The listing builds one solid part. Answer for the finished solid, in the listing's coordinates (mm). A direction names the side the tool comes from. Give positions to 0.01 mm unless a question says otherwise; leave off trailing zeros. Order: outer loops, then holes, each group sorted by start corner. A loop starts at its lowest first (then second) coordinate and runs counter-clockwise, first axis right, second up. Notation, with made-up numbers: (-17.5, -38.5) -> (17.5, -38.5) arc R16 cw to (17.5, -18.5) -> close; hole circle Ø11 at (19, 28.25). An arc over 180 degrees is marked (long way). Answer as a JSON object with one key per item and string values. Group by question number.
```python
from build123d import *

# Parameters (mm, degrees)
HOUSING_BODY_SKETCH_R   = 40
HOUSING_BODY_SKETCH_R_2 = 28
HOUSING_BODY_DEPTH      = 30
MOUNTING_FLANGE_DEPTH   = 25
KEYED_START             = 100
KEYED_HUB_SKETCH_R      = 28
KEYED_HUB_56_DEPTH      = 20
SIDE_RIB_DEPTH          = 20
SLOT_CUT_SKETCH_W       = 30
SLOT_CUT_SKETCH_H       = 10
SLOT_CUT_10X30_DEPTH    = 118.08543889


with BuildPart() as part:
    # Housing Body Sketch → Housing Body (new, symmetric)
    with BuildSketch(Plane(origin=(0, 0, 0), x_dir=(0, 0, -1), z_dir=(1, 0, 0))):
        Circle(HOUSING_BODY_SKETCH_R)
        Circle(HOUSING_BODY_SKETCH_R_2, mode=Mode.SUBTRACT)
    extrude(amount=HOUSING_BODY_DEPTH, both=True)

    # Mounting Flange Sketch → Mounting Flange (add, symmetric)
    with BuildSketch(Plane(origin=(0, 0, 0), x_dir=(0, 0, -1), z_dir=(1, 0, 0))):
        with BuildLine():
            Line((-33.071891388, -22.5), (-50, -22.5))
            Line((-50, -22.5), (-50, -53))
            Line((-50, -53), (50, -53))
            Line((50, -53), (50, 53))
            Line((50, 53), (-50, 53))
            Line((-50, 53), (-50, 22.5))
            Line((-50, 22.5), (-33.071891388, 22.5))
            ThreePointArc((-33.071891388, 22.5), (11.771243445, 38.228756555), (40, 0))
            ThreePointArc((40, 0), (11.771243445, -38.228756555), (-33.071891388, -22.5))
        make_face()
    extrude(amount=MOUNTING_FLANGE_DEPTH, both=True)



with BuildPart() as body_2:
    # Keyed Hub Sketch → Keyed Hub Ø56 (new body)
    with BuildSketch(Plane.XY.offset(KEYED_START)):
        Circle(KEYED_HUB_SKETCH_R)
        with BuildLine():
            Line((-4, 12.369316877), (-4, 15.369316877))
            Line((-4, 15.369316877), (4, 15.369316877))
            Line((4, 15.369316877), (4, 12.369316877))
            ThreePointArc((4, 12.369316877), (0, -13), (-4, 12.369316877))
        make_face(mode=Mode.SUBTRACT)
    extrude(amount=-KEYED_HUB_56_DEPTH)


with BuildPart() as part_1:
    add(part.part)

    add(body_2.part)  # Side Rib merges body 2
    # Side Rib Sketch → Side Rib (add, symmetric)
    with BuildSketch(Plane(origin=(0, 0, 0), x_dir=(0, 0, -1), z_dir=(1, 0, 0))):
        Polygon((-50, 35), (-95, 35), (-95, 17), (-80, 17), (-80, 22.5), (-50, 22.5), align=None)
    side_rib = extrude(amount=SIDE_RIB_DEPTH, both=True)

    # Side Rib Mirror: Side Rib across plane
    add(side_rib.mirror(Plane.ZX))

    # Slot Cut Sketch → Slot Cut 10x30 (cut, through all)
    with BuildSketch(Plane.XY.offset(50)):
        with Locations((0, 48)):
            Rectangle(SLOT_CUT_SKETCH_W, SLOT_CUT_SKETCH_H)
    slot_cut_10x30 = extrude(amount=-SLOT_CUT_10X30_DEPTH, mode=Mode.SUBTRACT)

    # Slot Cut Mirror: Slot Cut 10x30 across plane
    add(slot_cut_10x30.mirror(Plane.ZX), mode=Mode.SUBTRACT)


solid = part_1.part
```
(1) A cutting plane is placed at D-D (y = 18). Determine the outline of the cut face in (x, z), and give its area (3 significant figures).
(2) Find the intervals of material crossed by line 1 along X through (y, z) = (0, 86); line 2 along Z through (x, y) = (-9, -19.5); line 3 along Y through (x, z) = (-11, 57.5), in increasing order. Write a range as [from, to].
(3) Flat-ended cylindrical pins translate along their axes: pin 1 Ø2 at (x, z) = (15.5, 60) entering from -Y; pin 2 Ø15 at (x, z) = (5.5, 13.5) entering from +Y; pin 3 Ø24 at (x, z) = (-2, 6) entering from -Y. Find the tip coordinate at first contact, or state that the pin passes through.
(4) A cutting plane is placed at A-A (y = 0). Determine the outline of the cut face in (x, z), and give its area (3 significant figures).
(5) Which of the six approach directions +Z, -Z, +X, -X, +Y, -Y give full straight-line access (tool end or side, diameter ignored) to faces 1 (the flat face through (0, 43, 1)), 2 (the flat face through (-15, -48, 1)), 3 (the flat face through (0, 31, 95)), 4 (the flat face through (0, -22.5, 57)), 5 (the flat face through (4, 14, 90))?
(6) A cutting plane is placed at C-C (x = 0). Determine the outline of the cut face in (y, z).
(7) For a pull along Y with two mould halves and no side action, classify faces 6 (the flat face through (-20, -53, 1)), 7 (the cylindrical face through (-27.973, 1.231, 92.362)), 8 (the flat face through (-4, 14, 90)), 9 (the flat face through (-30, -8, 27)) as +Y half, -Y half, draft (parallel to the pull), parting line (faces both ways), or undercut.
(8) A cutting plane is placed at B-B (z = 54). Determine the outline of the cut face in (x, y), and give its area (3 significant figures).
Check sheet entries:
{
 "1": {"outline": "(-30, -35.72) -> (-25, -35.72) -> (-25, -50) -> (25, -50) -> (25, -35.72) -> (30, -35.72) -> (30, -21.45) -> (-30, -21.45) -> close; (-30, 21.45) -> (30, 21.45) -> (30, 35.72) -> (-30, 35.72) -> close; (-21.45, 80) -> (21.45, 80) -> (21.45, 100) -> (-21.45, 100) -> close", "area": "3,280 mm2"},
 "2": {"line 1": "x = [-28, -13], [13, 28]", "line 2": "z = [-50, -20.09], [20.09, 34.92], [80, 100]", "line 3": "y = [-35, -22.5], [22.5, 35]"},
 "3": {"pin 1": "stops at y = -35", "pin 2": "stops at y = 43", "pin 3": "stops at y = -43"},
 "4": {"outline": "(-30, -40) -> (-25, -40) -> (-25, -50) -> (25, -50) -> (25, -40) -> (30, -40) -> (30, -28) -> (-30, -28) -> close; (-30, 28) -> (30, 28) -> (30, 40) -> (-30, 40) -> close; (-28, 80) -> (-13, 80) -> (-13, 100) -> (-28, 100) -> close; (13, 80) -> (28, 80) -> (28, 100) -> (13, 100) -> close", "area": "2,540 mm2"},
 "5": {"face 1": "+Z, -Z, +Y", "face 2": "+Z, -Z, -Y", "face 3": "+Z, +Y", "face 4": "+X, -X", "face 5": "+Z"},
 "6": {"outline": "(-43, -50) -> (43, -50) -> (43, 50) -> (35, 50) -> (35, 95) -> (28, 95) -> (28, 100) -> (15.37, 100) -> (15.37, 80) -> (22.5, 80) -> (22.5, 33.07) arc R40 ccw to (-22.5, 33.07) -> (-22.5, 80) -> (-13, 80) -> (-13, 100) -> (-28, 100) -> (-28, 95) -> (-35, 95) -> (-35, 50) -> (-43, 50) -> close; hole circle Ø56 at (0, 0)"},
 "7": {"face 6": "-Y half", "face 7": "parting line", "face 8": "undercut", "face 9": "draft"},
 "8": {"outline": "(-20, -35) -> (20, -35) -> (20, -22.5) -> (-20, -22.5) -> close; (-20, 22.5) -> (20, 22.5) -> (20, 35) -> (-20, 35) -> close", "area": "1,000 mm2"}
}
